The model under review builds one solid part; all positions refer to its coordinate system, in mm. Round coordinates to 2 decimals unless told otherwise and drop trailing zeros. Write each loop counter-clockwise with the first axis right and the second up, starting at its lowest first coordinate (ties: lowest second). Pieces come first, ordered by that corner, then holes. Notation, with made-up numbers: (13.25, 34) -> (27.25, 34) arc R31 cw to (27.25, 60) -> close; hole circle Ø5 at (84.25, 23). An arc over 180 degrees is marked (long way). Use CSV: the item, a comma, the result in double quotes. Start each with the question number.
1) Take a section at C-C, the plane y = 2.5. State how many separate pieces and enclosed holes the cut face has, then the cut area to 3 significant figures.
2) Mouldability with a two-part tool opening along X and no side actions: class faces 1 (the face through (-104, 5, 326)), 2 (the face through (-206.9, -0.1, -269.8)), 3 (the face through (21.984, 0.07, -499.516)) as released by +X, released by -X, zero draft, split by the parting line, or undercut.
3) For pin 1 Ø3 at (x, y) = (-351.5, -1.5) entering from -Z; pin 2 Ø6 at (x, y) = (-144, -1.5) entering from -Z; pin 3 Ø12 at (x, z) = (-415.75, 172.21) entering from +Y, all flat-tipped, find the tip position at first contact; note any pin that passes through.
4) Take a section at B-B, the plane x = 0. Give the boundary of the cut face in (y, z), then the cut area to 3 significant figures.
5) Wall thickness on probe 1 along X at (y, z) = (0, -13); probe 2 along Z at (x, y) = (-83.5, 2.75); probe 3 along Z at (x, y) = (115, -1): over which ranges is each line inside the solid? List them lowest first. Write a range as [from, to].
6) Take a section at D-D, the plane z = 386. Give the boundary of the cut face in (x, y), then the cut area to 3 significant figures.
7) Take a section at A-A, the plane z = 0. Give the boundary of the cut face in (x, y), then the cut area to 3 significant figures.
from build123d import *

# Parameters (mm, degrees)
SKETCH1_R                    = 500
SKETCH1_R_2                  = 340
BOSS_EXTRUDE1_DEPTH          = 5
F_13_5_13_5_DIAMETER_HOLE1_D = 13.5


with BuildPart() as part:
    # Sketch1 → Boss-Extrude1 (new, symmetric)
    with BuildSketch(Plane(origin=(0, 0, 0), x_dir=(1, 0, 0), z_dir=(0, 1, 0))):
        with Locations(Location((0, 0, 0), (0, 0, 270))):
            Circle(SKETCH1_R)
        with Locations(Location((0, 0, 0), (0, 0, 270))):
            Circle(SKETCH1_R_2, mode=Mode.SUBTRACT)
    extrude(amount=BOSS_EXTRUDE1_DEPTH, both=True)

    # Ø13.5 (13.5) Diameter Hole1 (through all)
    with Locations(Plane(origin=(0, 5, 0), x_dir=(1, 0, 0), z_dir=(0, 1, 0))):
        with Locations((172.207544564, 415.74578963), (415.74578963, 172.207544564), (415.74578963, -172.207544564), (172.207544564, -415.74578963), (-172.207544564, -415.74578963), (-415.74578963, -172.207544564), (-415.74578963, 172.207544564), (-172.207544564, 415.74578963)):
            Hole(F_13_5_13_5_DIAMETER_HOLE1_D / 2)


solid = part.part
Values found:
1,separate pieces,"1"
1,enclosed holes,"9"
1,area,"421,000 mm²"
2,face 1,"zero draft"
2,face 2,"undercut"
2,face 3,"split by the parting line"
3,pin 1,"z = -357.07"
3,pin 2,"z = -479.71"
3,pin 3,"through"
4,outline,"(-5, -500) -> (5, -500) -> (5, -340) -> (-5, -340) -> close; (-5, 340) -> (5, 340) -> (5, 500) -> (-5, 500) -> close"
4,area,"3,200 mm²"
5,probe 1,"[-499.83, -339.75], [339.75, 499.83]"
5,probe 2,"[-492.98, -329.59], [329.59, 492.98]"
5,probe 3,"[-486.6, -319.96], [319.96, 486.6]"
6,outline,"(-317.81, -5) -> (317.81, -5) -> (317.81, 5) -> (-317.81, 5) -> close"
6,area,"6,360 mm²"
7,outline,"(-500, -5) -> (-340, -5) -> (-340, 5) -> (-500, 5) -> close; (340, -5) -> (500, -5) -> (500, 5) -> (340, 5) -> close"
7,area,"3,200 mm²"
